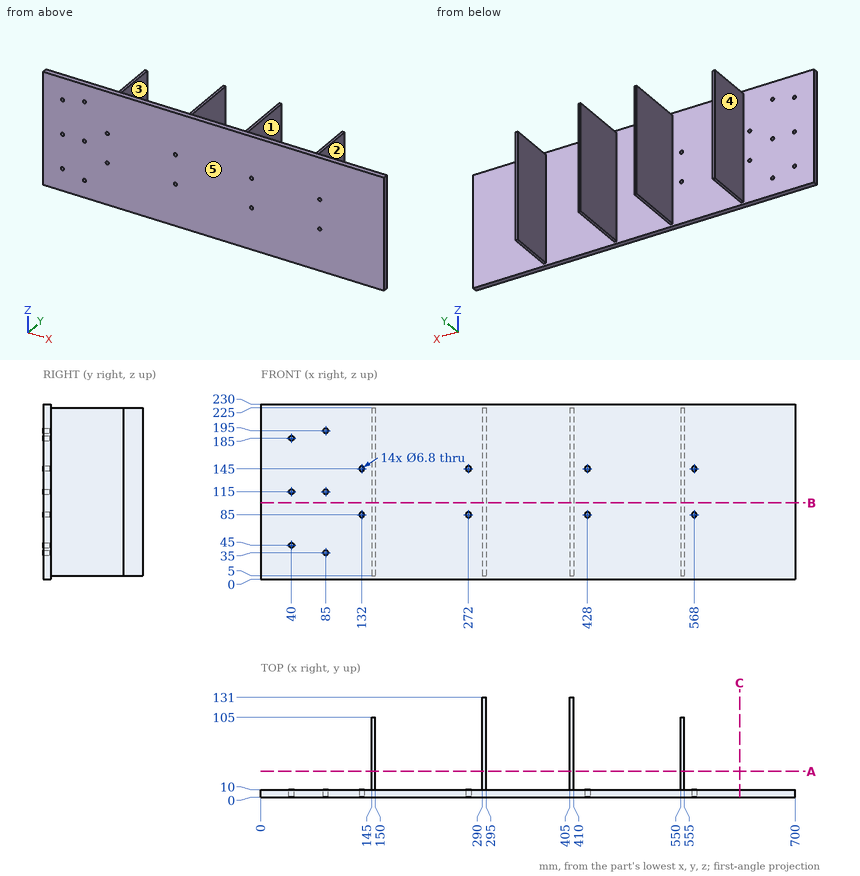
The drawing under review shows one solid part. Ordinate dimensions are in mm from its lowest x, y, z. A direction names the side the tool comes from. Give positions to 0.01 mm unless a question says otherwise; leave off trailing zeros. Order: outer loops, then holes, each group sorted by start corner. A loop starts at its lowest first (then second) coordinate and runs counter-clockwise, first axis right, second up. Notation, with made-up numbers: (-1, -9.75) - (48, -9.75) arc R6 cw to (48, 1.25) - close; hole circle Ø8 at (-31.75, 13). An arc over 180 degrees is marked (long way). Answer as a JSON object with one key per item and string values. Group by question number.
Item 1: Clearance check with flat-ended pins moving along their axes: pin 1 Ø4 at (x, z) = (92, 86.5) entering from +Y; pin 2 Ø2.5 at (x, y) = (293, 76) entering from +Z; pin 3 Ø2.5 at (x, z) = (146.5, 77) entering from +Y. State where each tip first meets the part, or that it passes through.
Item 2: Draft analysis for pull direction X (two halves, no side actions). For the marked faces 3, 4 and 5, state which applies: pulls with the +X half, pulls with the -X half, needs draft (parallel to the pull), parting line crosses it, or undercut.
Item 3: Take a section at B-B on z = 100.5. Give the boundary of the cut face in (x, y).
Item 4: Take a section at A-A on y = 34. Give the boundary of the cut face in (x, z).
Item 5: Wall thickness on line 1 along Z through (x, y) = (132, 5.5); line 2 along X through (y, z) = (6.5, 145); line 3 along X through (y, z) = (4.5, 115): over which ranges is each line inside the solid? List them lowest first.
Item 6: Machinability: for the marked faces 1 and 2, which of the approach directions +Z, -Z, +X, -X, +Y, -Y give a long, thin tool a straight path to every point of the face, cutting with its end or side? Answer none if there is none.
Item 7: Take a section at C-C on x = 627.5. Give the boundary of the cut face in (y, z), and give its area (3 significant figures).
Reported:
{
 "1": {"pin 1": "y = 10", "pin 2": "z = 225", "pin 3": "y = 105"},
 "2": {"face 3": "undercut", "face 4": "pulls with the -X half", "face 5": "needs draft"},
 "3": {"outline": "(0, 0) - (700, 0) - (700, 10) - (555, 10) - (555, 105) - (550, 105) - (550, 10) - (410, 10) - (410, 131) - (405, 131) - (405, 10) - (295, 10) - (295, 131) - (290, 131) - (290, 10) - (150, 10) - (150, 105) - (145, 105) - (145, 10) - (0, 10) - close"},
 "4": {"outline": "(145, 5) - (150, 5) - (150, 225) - (145, 225) - close; (290, 5) - (295, 5) - (295, 225) - (290, 225) - close; (405, 5) - (410, 5) - (410, 225) - (405, 225) - close; (550, 5) - (555, 5) - (555, 225) - (550, 225) - close"},
 "5": {"line 1": "0 to 81.6, 88.4 to 141.6, 148.4 to 230", "line 2": "0 to 128.6, 135.4 to 268.6, 275.4 to 424.6, 431.4 to 564.6, 571.4 to 700", "line 3": "0 to 36.6, 43.4 to 81.6, 88.4 to 700"},
 "6": {"face 1": "+Z, -Z, +Y", "face 2": "+Z, -Z, +X, +Y"},
 "7": {"outline": "(0, 0) - (10, 0) - (10, 230) - (0, 230) - close", "area": "2,300 mm^2"}
}
